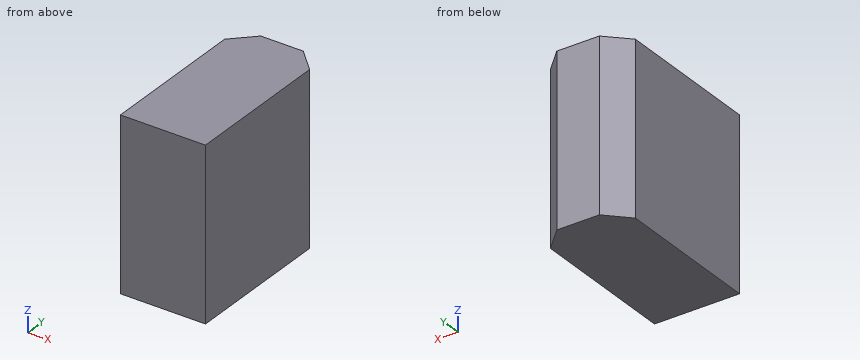
```python
from build123d import *

# Parameters (mm, degrees)
SKETCH1_W           = 20
SKETCH1_H           = 40
BOSS_EXTRUDE1_DEPTH = 40
CHAMFER1_SIZE       = 5


with BuildPart() as part:
    # Sketch1 → Boss-Extrude1 (new body)
    with BuildSketch(Plane.XY):
        Rectangle(SKETCH1_W, SKETCH1_H)
    extrude(amount=BOSS_EXTRUDE1_DEPTH)

    # Chamfer1
    chamfer1_edges = [part.edges().sort_by_distance(p)[0] for p in [
        (-10, 20, 20),
        (10, 20, 20),
    ]]
    chamfer(chamfer1_edges, length=CHAMFER1_SIZE)


solid = part.part
```
Source: CAD feature listing. Evaluate the final solid. Frame: model axes, mm. Give positions to 0.01 mm unless a question says otherwise; leave off trailing zeros. Loops run counter-clockwise (first coordinate to the right, second up) from the corner with the lowest first, then second, coordinate; pieces in that order, holes last. Notation, with made-up numbers: (47.25, 79.5) -> (67.25, 79.5) arc R29 cw to (67.25, 110.5) -> close; hole circle Ø11 at (-32.5, 46.5). An arc over 180 degrees is marked (long way). Use a Markdown table: item, result. Add a question column.
(1) Section query B-B (x = -7.75). Output: boundary loops of the cut face in (y, z).
(2) Section query A-A (z = 14). Output: boundary loops of the cut face in (x, y).
(3) Section query C-C (x = 8). Output: boundary loops of the cut face in (y, z), then the cut area to 3 significant figures.
(4) Ray query, line 1 (Y direction, x = -6, z = 19.5); line 2 (X direction, y = 17, z = 26.5); line 3 (Y direction, x = -8, z = 4). Return the intervals inside material, ascending.
Checked values:
| question | item | result |
|---|---|---|
| 1 | outline | (-20, 0) -> (17.25, 0) -> (17.25, 40) -> (-20, 40) -> close |
| 2 | outline | (-10, -20) -> (10, -20) -> (10, 15) -> (5, 20) -> (-5, 20) -> (-10, 15) -> close |
| 3 | outline | (-20, 0) -> (17, 0) -> (17, 40) -> (-20, 40) -> close |
| 3 | area | 1,480 mm^2 |
| 4 | line 1 | -20 to 19 |
| 4 | line 2 | -8 to 8 |
| 4 | line 3 | -20 to 17 |
